from build123d import *

# Parameters (mm, degrees)
BASEKEY_DEPTH = 4
CHAMFER1_SIZE = 0.6


with BuildPart() as part:
    # Sketch1 → BaseKey (new, symmetric)
    with BuildSketch(Plane.XY):
        with BuildLine():
            Line((-15, 5), (0, 5))
            ThreePointArc((0, 5), (5, 0), (0, -5))
            Line((0, -5), (-15, -5))
            ThreePointArc((-15, -5), (-20, 0), (-15, 5))
        make_face()
    extrude(amount=BASEKEY_DEPTH, both=True)

    # Chamfer1
    chamfer1_edges = [part.edges().sort_by_distance(p)[0] for p in [
        (5, 0, 4),
        (-7.5, 5, 4),
        (-20, 0, 4),
        (-7.5, 5, -4),
        (5, 0, -4),
        (-7.5, -5, -4),
        (-20, 0, -4),
        (-7.5, -5, 4),
    ]]
    chamfer(chamfer1_edges, length=CHAMFER1_SIZE)


solid = part.part
Build history of the part. All positions in model axes, mm. Give positions to 0.01 mm unless a question says otherwise; leave off trailing zeros. Order: outer loops, then holes, each group sorted by start corner. A loop starts at its lowest first (then second) coordinate and runs counter-clockwise, first axis right, second up. Notation, with made-up numbers: M -3,59.25 L 2,59.25 A17 cw 2,87.25 Z; hole C 34,-8.5 d7. An arc over 180 degrees is marked long. Put each result on its own line as item: value.
Item 1: Slice it at A-A, the plane z = 0.5. Write the cut outline in (x, y), plus the area to 3 significant figures.
From the geometry:
outline: M -15,-5 L 0,-5 A5 ccw 0,5 L -15,5 A5 ccw Z
area: 229 mm2
Item 2: Flat gauge pin, fed straight in: pin 1 Ø1.5 at (x, z) = (1, -0.5) entering from +Y. Where does the tip first touch, or does it go through?
From the geometry:
pin 1: stops at y = 4.99
Item 3: Probe line 1 (X direction, y = -1, z = -2.25); line 2 (Y direction, x = -16.25, z = -0.25); line 3 (X direction, y = 3, z = 1). List the from-to ranges inside material, lowest first. Write a range as [from, to].
From the geometry:
line 1: x = [-19.9, 4.9]
line 2: y = [-4.84, 4.84]
line 3: x = [-19, 4]
